Source: CAD feature listing. Evaluate the final solid. Frame: model axes, mm. Face numbers are marked on the shaded views. Coordinates: 2 decimals unless noted, no trailing zeros. Write each loop counter-clockwise with the first axis right and the second up, starting at its lowest first coordinate (ties: lowest second). Pieces come first, ordered by that corner, then holes. Notation, with made-up numbers: M -13,52.25 L -4,52.25 A15 ccw -4,78.25 Z; hole C -13,7.25 d2. An arc over 180 degrees is marked long. Answer as CSV lines item,"result". Start each with the question number.
1. Mould query, pull axis X, two halves, no side actions, for the marked faces 1, 2, 3 and 4. Classes: pulls with the +X half, pulls with the -X half, needs draft (parallel to the pull), parting line crosses it, or undercut.
2. Section C-C on z = 5.55. Return the cut outline in (x, y) (3 decimals).
3. Section D-D on x = -3.5. Return the cut outline in (y, z).
4. Line query: probe 1 along X at (y, z) = (0, 1.8); probe 2 along Y at (x, z) = (3.5, 2.8); probe 3 along X at (y, z) = (0.25, 5.55). Output: solid intervals per line, ascending. Write a range as [from, to].
5. Section B-B on y = -5.25. Return the cut outline in (x, z), plus the area to 3 significant figures.
6. Section A-A on z = 2.6. Return the cut outline in (x, y), plus the area to 3 significant figures.
7. Contact query for flat-ended pins moving along their axis: pin 1 Ø2 at (x, z) = (-1.5, 0.5) entering from +Y; pin 2 Ø4 at (x, y) = (0.91, 0.75) entering from -Z; pin 3 Ø1 at (x, z) = (3.5, 1) entering from -Y; pin 4 Ø3 at (y, z) = (6, 4.5) entering from +X. Output: stop coordinate, or through.
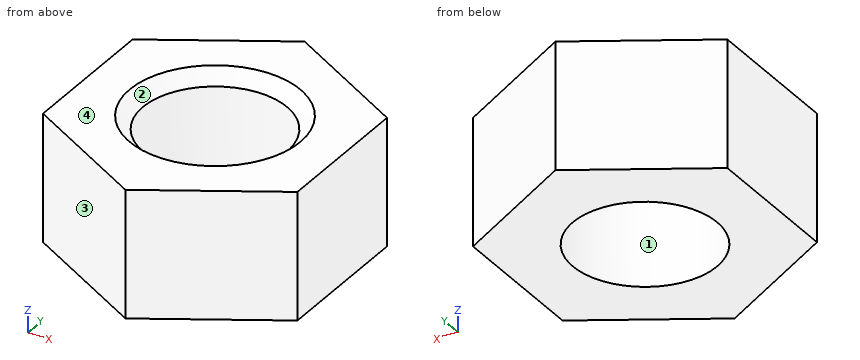
```python
from build123d import *

# Parameters (mm, degrees)
BOSS_EXTRUDE1_DEPTH         = 6
M8_TAPPED_HOLE1_D           = 6.8
M8_TAPPED_HOLE1_CSINK_D     = 8.05
M8_TAPPED_HOLE1_CSINK_ANGLE = 90


with BuildPart() as part:
    # Sketch1 → Boss-Extrude1 (new body)
    with BuildSketch(Plane.XY):
        Polygon((-5.093902669, -2.715310597), (-5.093902669, 4.212892633), (0.906097331, 7.676994248), (6.906097331, 4.212892633), (6.906097331, -2.715310597), (0.906097331, -6.179412212), align=None)
    extrude(amount=BOSS_EXTRUDE1_DEPTH)

    # M8 Tapped Hole1 (through all)
    with Locations(Plane.XY.offset(6)):
        with Locations((0.906097331, 0.748791018)):
            CounterSinkHole(M8_TAPPED_HOLE1_D / 2, M8_TAPPED_HOLE1_CSINK_D / 2, counter_sink_angle=M8_TAPPED_HOLE1_CSINK_ANGLE)


solid = part.part
```
Values:
1,face 1,"undercut"
1,face 2,"undercut"
1,face 3,"pulls with the -X half"
1,face 4,"needs draft"
2,outline,"M -5.094,-2.715 L 0.906,-6.179 L 6.906,-2.715 L 6.906,4.213 L 0.906,7.677 L -5.094,4.213 Z; hole C 0.906,0.749 d7.15"
3,outline,"M -3.64,0 L 5.13,0 L 5.13,6 L -3.64,6 Z"
4,probe 1,"[-5.09, -2.41], [4.22, 6.91]"
4,probe 2,"[-4.68, -1.45], [2.95, 6.18]"
4,probe 3,"[-5.09, -2.63], [4.45, 6.91]"
5,outline,"M -0.7,0 L 2.52,0 L 2.52,6 L -0.7,6 Z"
5,area,"19.3 mm²"
6,outline,"M -5.09,-2.72 L 0.91,-6.18 L 6.91,-2.72 L 6.91,4.21 L 0.91,7.68 L -5.09,4.21 Z; hole C 0.91,0.75 d6.8"
6,area,"88.4 mm²"
7,pin 1,"y = 6.87"
7,pin 2,"through"
7,pin 3,"y = -4.97"
7,pin 4,"x = 6.41"
